```python
from build123d import *

# Parameters (mm, degrees)
BOSS_EXTRUDE1_DEPTH = 7.5
SKETCH3_R           = 1.3
BOSS_EXTRUDE2_DEPTH = 10
CHAMFER1_SIZE       = 1


with BuildPart() as part:
    # Model → Boss-Extrude1 (new, symmetric)
    with BuildSketch(Plane.XY):
        Polygon((-51.414562431, 5.775101607), (-51.414562431, 20.775101607), (-70.671536853, 20.775099073), (-89.414562431, 20.775100292), (-89.414562431, 15.775100292), (-89.414562431, 12.775100292), (-70.671536853, 12.775100292), (-70.671536853, 5.775101607), (-70.671536853, -5.572423542), (-51.414562431, -5.572423542), align=None)
    extrude(amount=BOSS_EXTRUDE1_DEPTH, both=True)

    # Sketch3 → Boss-Extrude2 (add)
    with BuildSketch(Plane(origin=(-51.414562431, 0, 0), x_dir=(0, 0, -1), z_dir=(1, 0, 0))):
        with Locations(Location((-5, 3.217576458, 0), (0, 0, 270))):
            Circle(SKETCH3_R)
    extrude(amount=BOSS_EXTRUDE2_DEPTH)

    # Chamfer1
    chamfer1_edges = [part.edges().sort_by_distance(p)[0] for p in [
        (-80.043049642, 20.775099682, -7.5),
        (-61.043049642, 20.77510034, -7.5),
        (-51.414562431, 7.601339033, -7.5),
        (-61.043049642, -5.572423542, -7.5),
        (-70.671536853, 3.601338375, -7.5),
        (-80.043049642, 12.775100292, -7.5),
        (-61.043049642, -5.572423542, 7.5),
        (-51.414562431, 7.601339033, 7.5),
        (-89.414562431, 12.775100292, 0),
        (-89.414562431, 20.775100292, 0),
        (-51.414562431, 20.775101607, 0),
        (-51.414562431, -5.572423542, 0),
        (-70.671536853, -5.572423542, 0),
        (-61.043049642, 20.77510034, 7.5),
        (-80.043049642, 20.775099682, 7.5),
        (-89.414562431, 16.775100292, 7.5),
        (-80.043049642, 12.775100292, 7.5),
        (-70.671536853, 3.601338375, 7.5),
        (-89.414562431, 16.775100292, -7.5),
    ]]
    chamfer(chamfer1_edges, length=CHAMFER1_SIZE)


solid = part.part
```
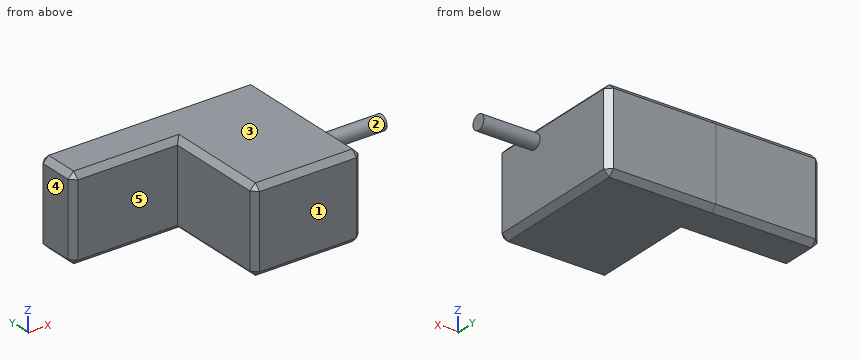
The listing builds one solid part. Answer for the finished solid, in the listing's coordinates (mm). Face numbers are marked on the shaded views. A direction names the side the tool comes from. Give positions to 0.01 mm unless a question says otherwise; leave off trailing zeros. Order: outer loops, then holes, each group sorted by start corner. A loop starts at its lowest first (then second) coordinate and runs counter-clockwise, first axis right, second up. Notation, with made-up numbers: (85.5, 39) - (136.5, 39) arc R22 cw to (136.5, 49) - close; hole circle Ø1 at (6, 45.5). An arc over 180 degrees is marked (long way). Answer in a Markdown table with one row per item. Add a question column.
Q1. Find the intervals of material crossed by line 1 along X through (y, z) = (8.75, -4.5); line 2 along Y through (x, z) = (-72, 5.25); line 3 along X through (y, z) = (19.75, -3.25), in increasing order. Write a range as [from, to].
Q2. The part is cut by section B-B (y = 14.75). Determine the outline of the cut face in (x, z), then the cut area to 3 significant figures.
Q3. Which of the six approach directions +Z, -Z, +X, -X, +Y, -Y give full straight-line access (tool end or side, diameter ignored) to the marked faces 4 and 5?
Q4. Given P1, Ø4, axis at y = 8, z = -2.5, coming from the -X side; P2, Ø4, axis at x = -77, z = 1, coming from the -Y side; P3, Ø5, axis at y = 13, z = -3.5, coming from the -X side; P4, Ø4, axis at y = -2.5, z = 2.5, coming from the +X side, each flat-ended and moving along its own axis, determine where each tip first touches the part or whether it passes through.
Q5. The part is cut by section C-C (x = -48.5). Determine the outline of the cut face in (y, z).
Q6. For a pull along Z with two mould halves and no side action, classify the marked faces 1, 2 and 3 as released by +Z, released by -Z, zero draft, split by the parting line, or undercut.
Q7. The part is cut by section A-A (z = 5). Determine the outline of the cut face in (x, y), then the cut area to 3 significant figures.
Q8. The part is cut by section D-D (z = -0.25). Determine the outline of the cut face in (x, y), then the cut area to 3 significant figures.
Determined:
| question | item | result |
|---|---|---|
| 1 | line 1 | x = [-70.67, -51.41] |
| 1 | line 2 | y = [12.78, 20.78] |
| 1 | line 3 | x = [-89.41, -51.41] |
| 2 | outline | (-89.41, -6.5) - (-88.41, -7.5) - (-52.41, -7.5) - (-51.41, -6.5) - (-51.41, 6.5) - (-52.41, 7.5) - (-88.41, 7.5) - (-89.41, 6.5) - close |
| 2 | area | 568 mm² |
| 3 | face 4 | +Z, -Z, -X, +Y, -Y |
| 3 | face 5 | +Z, -Z, -X, -Y |
| 4 | P1 | stops at x = -70.67 |
| 4 | P2 | stops at y = 12.78 |
| 4 | P3 | stops at x = -89.41 |
| 4 | P4 | stops at x = -51.41 |
| 5 | outline | circle Ø2.6 at (3.22, 5) |
| 6 | face 1 | zero draft |
| 6 | face 2 | split by the parting line |
| 6 | face 3 | released by +Z |
| 7 | outline | (-89.41, 13.78) - (-88.41, 12.78) - (-70.67, 12.78) - (-70.67, -4.57) - (-69.67, -5.57) - (-52.41, -5.57) - (-51.41, -4.57) - (-51.41, 1.92) - (-41.41, 1.92) - (-41.41, 4.52) - (-51.41, 4.52) - (-51.41, 19.78) - (-52.41, 20.78) - (-70.67, 20.78) - (-88.41, 20.78) - (-89.41, 19.78) - close |
| 7 | area | 681 mm² |
| 8 | outline | (-89.41, 13.78) - (-88.41, 12.78) - (-70.67, 12.78) - (-70.67, -4.57) - (-69.67, -5.57) - (-52.41, -5.57) - (-51.41, -4.57) - (-51.41, 19.78) - (-52.41, 20.78) - (-70.67, 20.78) - (-88.41, 20.78) - (-89.41, 19.78) - close |
| 8 | area | 655 mm² |
